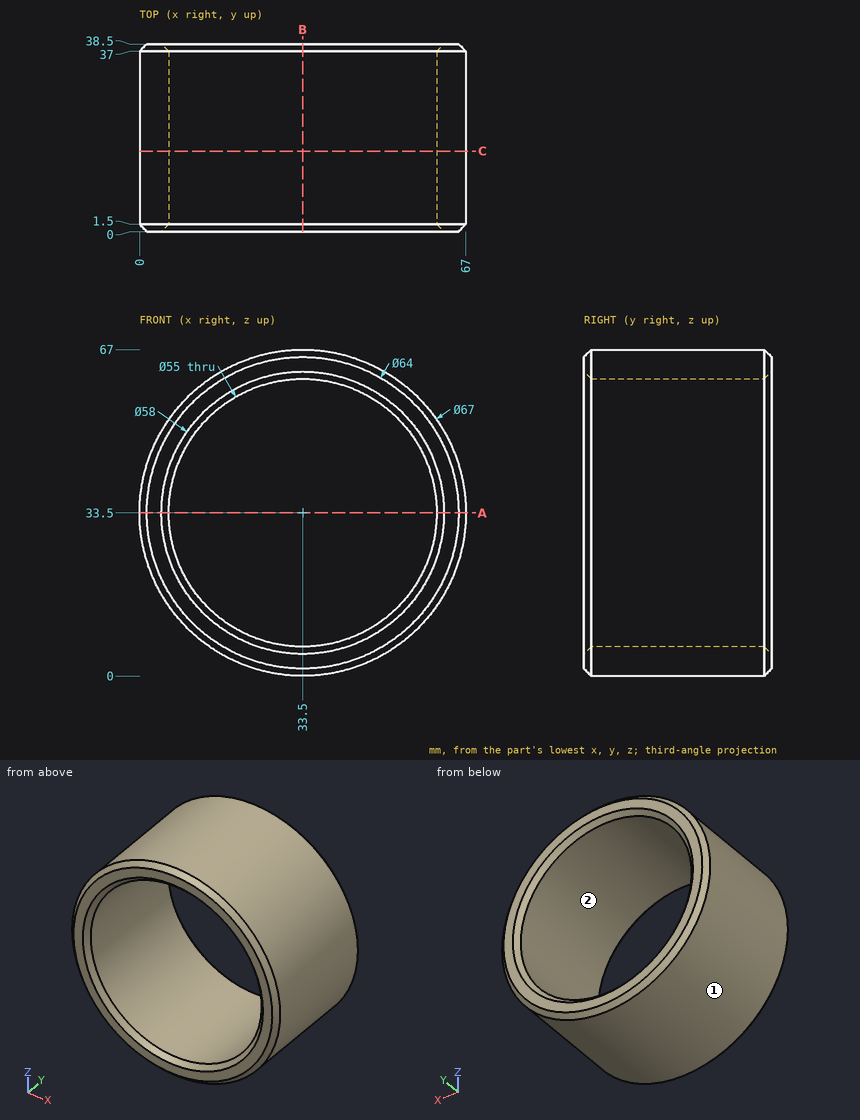
Could you check a few things on this drawing? It's one solid part, dimensions in mm from its lowest x, y, z. Round coordinates to 2 decimals unless told otherwise and drop trailing zeros. Order: outer loops, then holes, each group sorted by start corner. A loop starts at its lowest first (then second) coordinate and runs counter-clockwise, first axis right, second up. Notation, with made-up numbers: (49, 21) -> (104, 21) arc R9 cw to (104, 38) -> close; hole circle Ø5 at (7, 28). An arc over 180 degrees is marked (long way). One line per question, with ' | ' between items.
Q1. I'm going to push flat-ended pins straight in: pin 1 (1.5 mm diameter, centred on y = 29.5, z = 26, fed in from -X); pin 2 (1 mm diameter, centred on y = 23, z = 12, fed in from -X); pin 3 (1 mm diameter, centred on y = 17.5, z = 44.5, fed in from -X). Where does each tip first touch, or does it pass through?
Computed values:
pin 1: x = 0.69 | pin 2: x = 7.4 | pin 3: x = 1.69
Q2. If we section it at C-C on y = 16.5: Write out the boundary of the cut face in (x, z).
Computed values:
outline: circle Ø67 at (33.5, 33.5); hole circle Ø55 at (33.5, 33.5)
Q3. We'd pull the mould along Z, two halves only. Please class the marked faces 1 and 2: released by +Z, released by -Z, zero draft, split by the parting line, or undercut.
Computed values:
face 1: split by the parting line | face 2: undercut
Q4. If we section it at B-B on x = 33.5: Write out the boundary of the cut face in (y, z).
Computed values:
outline: (0, 1.5) -> (1.5, 0) -> (37, 0) -> (38.5, 1.5) -> (38.5, 4.5) -> (37, 6) -> (1.5, 6) -> (0, 4.5) -> close; (0, 62.5) -> (1.5, 61) -> (37, 61) -> (38.5, 62.5) -> (38.5, 65.5) -> (37, 67) -> (1.5, 67) -> (0, 65.5) -> close
Q5. If we section it at A-A on z = 33.5: Write out the boundary of the cut face in (x, y), plus the area to 3 significant figures.
Computed values:
outline: (0, 1.5) -> (1.5, 0) -> (4.5, 0) -> (6, 1.5) -> (6, 37) -> (4.5, 38.5) -> (1.5, 38.5) -> (0, 37) -> close; (61, 1.5) -> (62.5, 0) -> (65.5, 0) -> (67, 1.5) -> (67, 37) -> (65.5, 38.5) -> (62.5, 38.5) -> (61, 37) -> close | area: 453 mm²
Q6. If I drill on line 1 (Z direction, x = 32.5, y = 30); line 2 (X direction, y = 12, z = 33); line 3 (Z direction, x = 52, y = 15), over which ranges is the centre line in solid material (lowest first)? Write a range as from..to.
Computed values:
line 1: 0.01..6.02, 60.98..66.99 | line 2: 0..6, 61..67 | line 3: 5.57..13.15, 53.85..61.43
